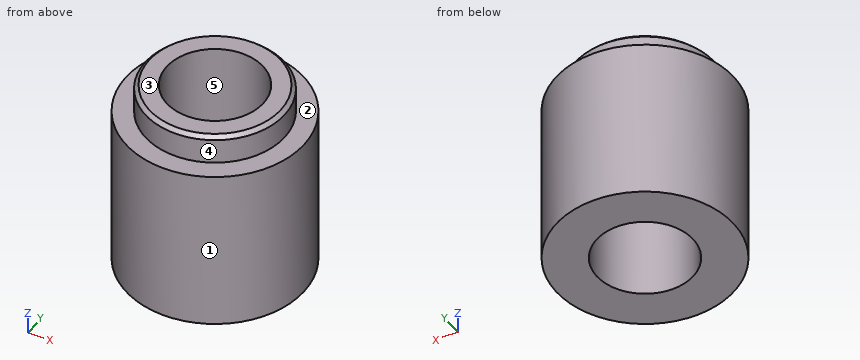
from build123d import *

# Parameters (mm, degrees)
SKETCH1_R           = 23
BOSS_EXTRUDE1_DEPTH = 50
CUT_EXTRUDE1_START  = -7.5
SKETCH2_R           = 23
SKETCH2_R_2         = 18
CUT_EXTRUDE1_DEPTH  = 7.5
SKETCH3_R           = 12.5
CUT_EXTRUDE2_DEPTH  = 60.648973168
CHAMFER1_SIZE       = 1


with BuildPart() as part:
    # Sketch1 → Boss-Extrude1 (new body)
    with BuildSketch(Plane.XY):
        Circle(SKETCH1_R)
    extrude(amount=BOSS_EXTRUDE1_DEPTH)

    # Sketch2 → Cut-Extrude1 (cut)
    with BuildSketch(Plane.XY.offset(50).offset(CUT_EXTRUDE1_START)):
        Circle(SKETCH2_R)
        Circle(SKETCH2_R_2, mode=Mode.SUBTRACT)
    extrude(amount=CUT_EXTRUDE1_DEPTH, mode=Mode.SUBTRACT)

    # Sketch3 → Cut-Extrude2 (cut, through all)
    with BuildSketch(Plane.XY.offset(50)):
        Circle(SKETCH3_R)
    extrude(amount=-CUT_EXTRUDE2_DEPTH, mode=Mode.SUBTRACT)

    # Chamfer1
    chamfer1_edges = [part.edges().sort_by_distance(p)[0] for p in [
        (-18, 0, 50),
    ]]
    chamfer(chamfer1_edges, length=CHAMFER1_SIZE)


solid = part.part
Check sheet for the modelled part. Datum: model origin and axes. Units: mm. Face numbers are marked on the shaded views. A direction names the side the tool comes from. Coordinates: 2 decimals unless noted, no trailing zeros. Loops run counter-clockwise (first coordinate to the right, second up) from the corner with the lowest first, then second, coordinate; pieces in that order, holes last. Notation, with made-up numbers: (69.5, 4.5) -> (76.5, 4.5) arc R28 cw to (76.5, 36.5) -> close; hole circle Ø11 at (-20, -6). An arc over 180 degrees is marked (long way). Write item = value, one per line. Start each with the question number.
1. Tool access check on the marked faces 1 and 2. Record the directions out of +Z, -Z, +X, -X, +Y, -Y that give a thin tool (end or side, any length) a straight path to the whole face; none if there is none.
2. Section check A-A on x = 0. Record the cut outline in (y, z), then the cut area to 3 significant figures.
3. Draft check along Y on the marked faces 3, 4 and 5. Enter one of: released by +Y, released by -Y, zero draft, split by the parting line, or undercut.
4. Material ranges on line 1 (Y direction, x = 0, z = 26); line 2 (Y direction, x = 4.5, z = 20); line 3 (X direction, y = 6, z = 33.5), recorded low to high.
5. Section check D-D on z = 46.5. Record the cut outline in (x, y).
6. Depth check by flat-ended pin: P1, Ø12, axis at x = -3, z = 38.5, coming from the -Y side; P2, Ø5, axis at y = 7.5, z = 43, coming from the -X side; P3, Ø5, axis at x = 14.5, y = 18, coming from the +Z side; P4, Ø22.5, axis at x = 0, y = 0, coming from the -Z side. Enter the tip coordinate at first touch or a pass-through.
7. Section check C-C on z = 5. Record the cut outline in (x, y).
Responses:
q1.face_1 = +Z, -Z
q1.face_2 = +Z
q2.outline = (-23, 0) -> (-12.5, 0) -> (-12.5, 50) -> (-17, 50) -> (-18, 49) -> (-18, 42.5) -> (-23, 42.5) -> close; (12.5, 0) -> (23, 0) -> (23, 42.5) -> (18, 42.5) -> (18, 49) -> (17, 50) -> (12.5, 50) -> close
q2.area = 974 mm2
q3.face_3 = zero draft
q3.face_4 = split by the parting line
q3.face_5 = undercut
q4.line_1 = -23 to -12.5, 12.5 to 23
q4.line_2 = -22.56 to -11.66, 11.66 to 22.56
q4.line_3 = -22.2 to -10.97, 10.97 to 22.2
q5.outline = circle Ø36 at (0, 0); hole circle Ø25 at (0, 0)
q6.P1 = -23
q6.P2 = -22.44
q6.P3 = 42.5
q6.P4 = through
q7.outline = circle Ø46 at (0, 0); hole circle Ø25 at (0, 0)
